CAD build for the part. Positions are in the model's coordinates, mm. A direction names the side the tool comes from. Give positions to 0.01 mm unless a question says otherwise; leave off trailing zeros. Loops run counter-clockwise (first coordinate to the right, second up) from the corner with the lowest first, then second, coordinate; pieces in that order, holes last.
Item 1: Saw through at A-A on x = 17. Give the cut face in (y, z).
Item 2: Drop flat-ended pins along their axis: P1, Ø3, axis at y = 0, z = 3.5, coming from the -X side; P2, Ø1.5, axis at x = 25, z = -3, coming from the -Y side; P3, Ø10, axis at x = 20, y = -6.5, coming from the +Z side; P4, Ø6, axis at x = 27.5, y = 7, coming from the +Z side. Give the stop position or say it passes through.
Item 3: Probe probe 1 along X at (y, z) = (-7.75, 0.5); probe 2 along Z at (x, y) = (8, 3.75); probe 3 along X at (y, z) = (-1.5, 5). List the from-to ranges inside material, lowest first.
Item 4: Which spindle directions (+Z, -Z, +X, -X, +Y, -Y) get a long thin tool onto all of the face, cutting with end or side? Do faces 1 (the flat face through (6.4, -4, -5)), 2 (the flat face through (51.4, 0, 0)). Say none if no direction does.
from build123d import *

# Parameters (mm, degrees)
BOSS_EXTRUDE1_DEPTH = 6.4
SKETCH4_R           = 17.59
SKETCH4_R_2         = 8
CUT_EXTRUDE1_DEPTH  = 0.8
CUT_EXTRUDE1_DRAFT  = -60
CHAMFER2_SIZE       = 0.555555556


with BuildPart() as part:
    # Sketch3 → Boss-Extrude1 (new body)
    with BuildSketch(Plane(origin=(0, 0, 0), x_dir=(0, 0, -1), z_dir=(1, 0, 0))):
        Polygon((8, 4.618802154), (0, 9.237604307), (-8, 4.618802154), (-8, -4.618802154), (0, -9.237604307), (8, -4.618802154), align=None)
    extrude(amount=BOSS_EXTRUDE1_DEPTH)


with BuildPart() as cut_extrude1_tool:
    # Sketch4 → Cut-Extrude1 (with draft: the straight prism first)
    with BuildSketch(Plane.ZY):
        Circle(SKETCH4_R)
        Circle(SKETCH4_R_2, mode=Mode.SUBTRACT)
    extrude(amount=-CUT_EXTRUDE1_DEPTH)
    # Cut-Extrude1: the draft: its side faces are tilted about the plane it starts from
    cut_extrude1_sides = [cut_extrude1_tool.faces().sort_by_distance(p)[0] for p in [
        (0.4, 0, -17.59),
        (0.4, 0, -8),
    ]]
    draft(cut_extrude1_sides, Plane.ZY, CUT_EXTRUDE1_DRAFT)


with BuildPart() as part_1:
    add(part.part)

    # Cut-Extrude1: cut by cut_extrude1_tool
    add(cut_extrude1_tool.part, mode=Mode.SUBTRACT)

    # Sketch5 → Revolve1 (revolve)
    with BuildSketch(Plane.XY, mode=Mode.PRIVATE) as revolve1_sk:
        with BuildLine():
            Line((7.5, 5), (51.4, 5))
            Line((51.4, 5), (51.4, 0))
            Line((51.4, 0), (6.4, 0))
            Line((6.4, 0), (6.4, 6.1))
            ThreePointArc((6.4, 6.1), (6.722182541, 5.322182541), (7.5, 5))
        make_face()
    revolve(revolve1_sk.sketch.rotate(Axis((6.4, 0, 0), (1, 0, 0)), 90), axis=Axis((6.4, 0, 0), (1, 0, 0)))

    # Chamfer2
    chamfer2_edges = [part_1.edges().sort_by_distance(p)[0] for p in [
        (51.4, 0, -5),
    ]]
    chamfer(chamfer2_edges, length=CHAMFER2_SIZE)


solid = part_1.part
Results below:
1. outline: circle Ø10 at (0, 0)
2. P1: stops at x = 0
2. P2: stops at y = -4.47
2. P3: stops at z = 4.77
2. P4: stops at z = 3
3. probe 1: x = 0 to 6.4
3. probe 2: z = -3.31 to 3.31
3. probe 3: x = 0 to 6.84
4. face 1: +X
4. face 2: +Z, -Z, +X, +Y, -Y
